Here's the drawing with two shaded views (mm, measured from the low corner). I have some questions. A direction names the side the tool comes from. Coordinates: 2 decimals unless noted, no trailing zeros. Loops run counter-clockwise (first coordinate to the right, second up) from the corner with the lowest first, then second, coordinate; pieces in that order, holes last. Notation, with made-up numbers: M 67.25,29 L 86.25,29 A23 cw 86.25,67 Z; hole C 61.5,64 d1. An arc over 180 degrees is marked long. Return JSON: item names as keys, results as strings. Group by question number.
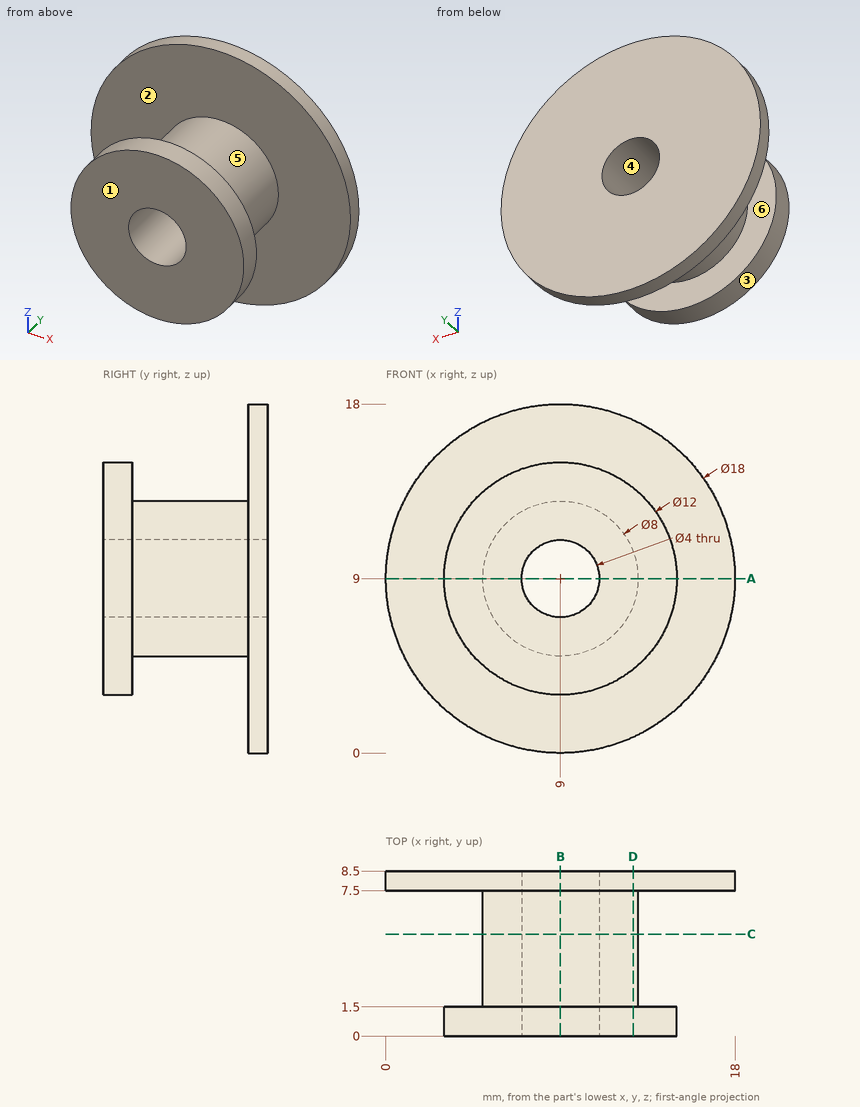
(1) For the marked faces 1, 2 and 3, which set-ups out of +Z, -Z, +X, -X, +Y, -Y let a thin tool reach every point of the face, with its end or its side?
(2) Imagine slicing it at C-C, the plane y = 5.25. Write out the boundary of the cut face in (x, z), then the cut area to 3 significant figures.
(3) If I drill on L1, parallel to X at y = 3, z = 9; L2, parallel to Y at x = 7.5, z = 4, over which ranges is the centre line in solid material (lowest first)? Write a range as [from, to].
(4) Will these pins go through, and if not, where does the flat tip stop? P1, Ø3, axis at y = 5, z = 6.5, coming from the +X side; P2, Ø2, axis at y = 1.5, z = 10.5, coming from the -X side; P3, Ø3, axis at x = 3.5, y = 2, coming from the -Z side.
(5) Imagine slicing it at D-D, the plane x = 12.75. Write out the boundary of the cut face in (y, z).
(6) Imagine slicing it at A-A, the plane z = 9. Write out the boundary of the cut face in (x, y), then the cut area to 3 significant figures.
(7) We'd pull the mould along X, two halves only. Please class the marked faces 4, 5 and 6: +X half, -X half, draft (parallel to the pull), parting line (faces both ways), or undercut.
(8) Imagine slicing it at B-B, the plane x = 9. Write out the boundary of the cut face in (y, z), then the cut area to 3 significant figures.
Checks:
{
 "1": {"face 1": "+Z, -Z, +X, -X, -Y", "face 2": "none", "face 3": "-Y"},
 "2": {"outline": "C 9,9 d8; hole C 9,9 d4", "area": "37.7 mm²"},
 "3": {"L1": "[5, 7], [11, 13]", "L2": "[0, 1.5], [7.5, 8.5]"},
 "4": {"P1": "x = 12.87", "P2": "x = 3.02", "P3": "z = 4.61"},
 "5": {"outline": "M 0,4.32 L 1.5,4.32 L 1.5,7.61 L 7.5,7.61 L 7.5,0.82 L 8.5,0.82 L 8.5,17.18 L 7.5,17.18 L 7.5,10.39 L 1.5,10.39 L 1.5,13.68 L 0,13.68 Z"},
 "6": {"outline": "M 0,7.5 L 5,7.5 L 5,1.5 L 3,1.5 L 3,0 L 7,0 L 7,8.5 L 0,8.5 Z; M 11,0 L 15,0 L 15,1.5 L 13,1.5 L 13,7.5 L 18,7.5 L 18,8.5 L 11,8.5 Z", "area": "50.0 mm²"},
 "7": {"face 4": "undercut", "face 5": "parting line", "face 6": "draft"},
 "8": {"outline": "M 0,3 L 1.5,3 L 1.5,5 L 7.5,5 L 7.5,0 L 8.5,0 L 8.5,7 L 0,7 Z; M 0,11 L 8.5,11 L 8.5,18 L 7.5,18 L 7.5,13 L 1.5,13 L 1.5,15 L 0,15 Z", "area": "50.0 mm²"}
}
